Can you work these out from the model? Positions are in its coordinate system, mm. A direction names the side the tool comes from. Round coordinates to 2 decimals unless told otherwise and drop trailing zeros. Order: outer loops, then holes, each group sorted by start corner. A loop starts at its lowest first (then second) coordinate and runs counter-clockwise, first axis right, second up. Notation, with made-up numbers: (82, -1) - (128, -1) arc R31 cw to (128, 35) - close; hole circle Ø3 at (27.5, -36.5). An arc over 180 degrees is marked (long way). Write item = value, one per line.
from build123d import *

# Parameters (mm, degrees)
BOSS_EXTRUDE1_DEPTH = 10
SHELL1_T            = -3


with BuildPart() as part:
    # Sketch2 → Boss-Extrude1 (new body)
    with BuildSketch(Plane.XY):
        with BuildLine():
            Line((0, 18), (-88, 18))
            ThreePointArc((-88, 18), (-106, 0), (-88, -18))
            Line((-88, -18), (0, -18))
            ThreePointArc((0, -18), (18, 0), (0, 18))
        make_face()
    extrude(amount=BOSS_EXTRUDE1_DEPTH)

    # Shell1
    shell1_openings = [part.faces().sort_by_distance(p)[0] for p in [
        (-44, 0, 10),
        (-44, 0, 0),
    ]]
    offset(amount=SHELL1_T, openings=shell1_openings, kind=Kind.INTERSECTION)


solid = part.part
(1) If we section it at C-C (z = 3): Write out the boundary of the cut face in (x, y).
Computed:
outline = (-88, -18) - (0, -18) arc R18 ccw to (0, 18) - (-88, 18) arc R18 ccw to start; hole (-88, -15) - (0, -15) arc R15 ccw to (0, 15) - (-88, 15) arc R15 ccw to start
(2) Will these pins go through, and if not, where does the flat tip stop? P1, Ø1.5, axis at y = -4, z = 6.5, coming from the -X side; P2, Ø6, axis at x = -88.5, z = 1, coming from the -Y side; P3, Ø1, axis at y = 7.5, z = 7, coming from the -X side; P4, Ø4, axis at y = -1, z = 9, coming from the +X side.
Computed:
P1 = -105.7
P2 = -18
P3 = -104.58
P4 = 18
(3) On a 3-axis mill with a long thin cutter (end or side, diameter ignored), from which of +Z, -Z, +X, -X, +Y, -Y can I reach the whole of each face in a straight line? I mean faces 1 (the face through (-43, 15, 5)), 2 (the face through (-106, 0, 5)). Say none if no direction works.
Computed:
face_1 = +Z, -Z
face_2 = +Z, -Z, -X
(4) If I drill on line 1 (Y direction, x = -75, z = 4.75); line 2 (Y direction, x = -95.5, z = 9.75); line 3 (X direction, y = -3, z = 3.25), over which ranges is the centre line in solid material (lowest first)? Write a range as from..to.
Computed:
line_1 = -18..-15, 15..18
line_2 = -16.36..-12.99, 12.99..16.36
line_3 = -105.75..-102.7, 14.7..17.75
(5) Thinking about a two-plate mould opening in Y: for faces 3 (the face through (-44, 16, 0)), 4 (the face through (-43, 18, 5)), 5 (the face through (-45, -15, 5)), which applies, +Y half, -Y half, draft (parallel to the pull), parting line (faces both ways), or undercut?
Computed:
face_3 = draft
face_4 = +Y half
face_5 = undercut
(6) If we section it at A-A (y = 0): Write out the boundary of the cut face in (x, z).
Computed:
outline = (-106, 0) - (-103, 0) - (-103, 10) - (-106, 10) - close; (15, 0) - (18, 0) - (18, 10) - (15, 10) - close
(7) If we section it at B-B (x = -53): Write out the boundary of the cut face in (y, z), plus the area to 3 significant figures.
Computed:
outline = (-18, 0) - (-15, 0) - (-15, 10) - (-18, 10) - close; (15, 0) - (18, 0) - (18, 10) - (15, 10) - close
area = 60.0 mm^2
